Input: part model. Units: mm. Frame: model coordinates. Face numbers are marked on the shaded views. A direction names the side the tool comes from. Coordinates: 2 decimals unless noted, no trailing zeros. Write each loop counter-clockwise with the first axis right and the second up, starting at its lowest first coordinate (ties: lowest second). Pieces come first, ordered by that corner, then holes. Notation, with made-up numbers: M 0.25,28.25 L 23.25,28.25 A18 cw 23.25,42.25 Z; hole C 25,85 d6. An arc over 180 degrees is marked long. Answer as a JSON object with one key per item and string values. Group by question number.
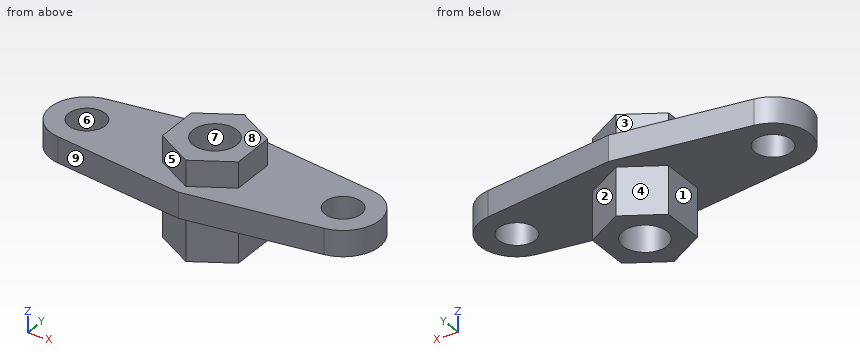
from build123d import *

# Parameters (mm, degrees)
LINK_PLATE_PROFILE_R  = 5
LINK_PLATE_DEPTH      = 3.5
FRONT_HEX_BOSS_DEPTH  = 10.5
REAR_HEX_BOSS_DEPTH   = 16.5
CENTRE_BORE_PROFILE_R = 6
CENTRE_BORE_12_DEPTH  = 72.572811156


with BuildPart() as part:
    # Link Plate Profile → Link Plate (new, symmetric)
    with BuildSketch(Plane.XY):
        with BuildLine():
            Line((55.952356647, 9.903324931), (19.565217391, 15))
            Line((19.565217391, 15), (-16.821921865, 9.903324931))
            ThreePointArc((-16.821921865, 9.903324931), (-25.434782609, 0), (-16.821921865, -9.903324931))
            Line((-16.821921865, -9.903324931), (19.565217391, -15))
            Line((19.565217391, -15), (55.952356647, -9.903324931))
            ThreePointArc((55.952356647, -9.903324931), (64.565217391, 0), (55.952356647, 9.903324931))
        make_face()
        with Locations((-15.434782609, 0)):
            Circle(LINK_PLATE_PROFILE_R, mode=Mode.SUBTRACT)
        Polygon((9.172912546, 6), (19.565217391, 12), (29.957522237, 6), (29.957522237, -6), (19.565217391, -12), (9.172912546, -6), align=None, mode=Mode.SUBTRACT)
        with Locations((54.565217391, 0)):
            Circle(LINK_PLATE_PROFILE_R, mode=Mode.SUBTRACT)
    extrude(amount=LINK_PLATE_DEPTH, both=True)

    # Front Hex Profile → Front Hex Boss (add)
    with BuildSketch(Plane.XY):
        Polygon((9.172912546, 6), (9.172912546, -6), (19.565217391, -12), (29.957522237, -6), (29.957522237, 6), (19.565217391, 12), align=None)
    extrude(amount=FRONT_HEX_BOSS_DEPTH)

    # Rear Hex Profile → Rear Hex Boss (add)
    with BuildSketch(Plane(origin=(0, 0, 0), x_dir=(-1, 0, 0), z_dir=(0, 0, -1))):
        Polygon((-9.172912546, 6), (-19.565217391, 12), (-29.957522237, 6), (-29.957522237, -6), (-19.565217391, -12), (-9.172912546, -6), align=None)
    extrude(amount=REAR_HEX_BOSS_DEPTH)

    # Centre Bore Profile → Centre Bore Ø12 (cut, through all)
    with BuildSketch(Plane.XY.offset(10.5)):
        with Locations((19.565217391, 0)):
            Circle(CENTRE_BORE_PROFILE_R)
    extrude(amount=-CENTRE_BORE_12_DEPTH, mode=Mode.SUBTRACT)


solid = part.part
Q1. Section B-B, the plane y = 0. Return the cut outline in (x, z).
Q2. Draft query along Y for the marked faces 6, 7, 8 and 9. Return one class per face: released by +Y, released by -Y, zero draft, split by the parting line, or undercut.
Q3. Section A-A, the plane z = -1.25. Return the cut outline in (x, y), and give its area (3 significant figures).
Q4. Access query for the marked faces 1, 2, 3, 4 and 5. Directions: +Z, -Z, +X, -X, +Y, -Y. A direction counts if a zero-diameter tool reaches every point of the face in a straight line with its end or side. Return the directions, or none.
Q5. Section D-D, the plane z = 5.75. Return the cut outline in (x, y).
Q6. Section C-C, the plane x = 17. Return the cut outline in (y, z).
Q7. Pin query (flat end, axial travel): pin 1 Ø13 at (x, y) = (54.57, 0) entering from -Z; pin 2 Ø3 at (x, z) = (23.5, -6.5) entering from +Y; pin 3 Ø3.5 at (y, z) = (2, 6.5) entering from +X; pin 4 Ø14 at (x, y) = (19.57, 0) entering from +Z. Return the tip coordinate at first contact, or that it passes through.
Q8. Line query: line 1 (Y direction, x = -13, z = -2.5); line 2 (Y direction, x = 55, z = 1); line 3 (Z direction, x = -21, y = 7). Output: solid intervals per line, ascending. Write a range as from..to.
Filled in:
{
 "1": {"outline": "M -25.43,-3.5 L -20.43,-3.5 L -20.43,3.5 L -25.43,3.5 Z; M -10.43,-3.5 L 9.17,-3.5 L 9.17,-16.5 L 13.57,-16.5 L 13.57,10.5 L 9.17,10.5 L 9.17,3.5 L -10.43,3.5 Z; M 25.57,-16.5 L 29.96,-16.5 L 29.96,-3.5 L 49.57,-3.5 L 49.57,3.5 L 29.96,3.5 L 29.96,10.5 L 25.57,10.5 Z; M 59.57,-3.5 L 64.57,-3.5 L 64.57,3.5 L 59.57,3.5 Z"},
 "2": {"face 6": "undercut", "face 7": "undercut", "face 8": "zero draft", "face 9": "released by -Y"},
 "3": {"outline": "M -16.82,-9.9 L 19.57,-15 L 55.95,-9.9 A10 ccw 55.95,9.9 L 19.57,15 L -16.82,9.9 A10 ccw Z; hole C -15.43,0 d10; hole C 19.57,0 d12; hole C 54.57,0 d10", "area": "1,800 mm^2"},
 "4": {"face 1": "-Z, -X, +Y, -Y", "face 2": "-Z, +X, +Y", "face 3": "+Z, -X, +Y", "face 4": "-Z, -X, +Y", "face 5": "+Z, -X, -Y"},
 "5": {"outline": "M 9.17,-6 L 19.57,-12 L 29.96,-6 L 29.96,6 L 19.57,12 L 9.17,6 Z; hole C 19.57,0 d12"},
 "6": {"outline": "M -14.64,-3.5 L -10.52,-3.5 L -10.52,-16.5 L -5.42,-16.5 L -5.42,10.5 L -10.52,10.5 L -10.52,3.5 L -14.64,3.5 Z; M 5.42,-16.5 L 10.52,-16.5 L 10.52,-3.5 L 14.64,-3.5 L 14.64,3.5 L 10.52,3.5 L 10.52,10.5 L 5.42,10.5 Z"},
 "7": {"pin 1": "z = -3.5", "pin 2": "y = 10.59", "pin 3": "x = 29.96", "pin 4": "z = 10.5"},
 "8": {"line 1": "-10.44..-4.37, 4.37..10.44", "line 2": "-10.04..-4.98, 4.98..10.04", "line 3": "-3.5..3.5"}
}
